Could you check a few things on this model? Use its own coordinates, in mm. A direction names the side the tool comes from. Give positions to 0.01 mm unless a question says otherwise; leave off trailing zeros. Order: outer loops, then holes, each group sorted by start corner. A loop starts at its lowest first (then second) coordinate and runs counter-clockwise, first axis right, second up. Notation, with made-up numbers: (64.25, 48) - (85.25, 48) arc R22 ccw to (85.25, 73) - close; hole circle Ø9 at (32, 82). An arc over 180 degrees is marked (long way). Put each result on its own line as item: value.
from build123d import *

# Parameters (mm, degrees)
CUT_EXTRUDE_START   = -15
CUT_EXTRUDE_1_DEPTH = 4
CHAMFER_1_SIZE      = 1


with BuildPart() as part:
    # 草图1 → 旋转1 (revolve)
    with BuildSketch(Plane.XY, mode=Mode.PRIVATE) as revolve_1_sk:
        Polygon((0, 0), (0, 15), (4.4, 15), (4.4, 14.3), (6, 14.3), (6, 15), (164, 15), (164, 20), (169, 20), (169, 0), align=None)
    revolve(revolve_1_sk.sketch.rotate(Axis((0, 0, 0), (1, 0, 0)), 90), axis=Axis((0, 0, 0), (1, 0, 0)))

    # 草图2 → 切除-拉伸1 (cut)
    with BuildSketch(Plane.XY.offset(CUT_EXTRUDE_START)):
        with BuildLine():
            Line((119, -4), (49, -4))
            ThreePointArc((49, -4), (45, 0), (49, 4))
            Line((49, 4), (119, 4))
            ThreePointArc((119, 4), (123, 0), (119, -4))
        make_face()
    extrude(amount=CUT_EXTRUDE_1_DEPTH, mode=Mode.SUBTRACT)

    # 倒角1
    chamfer_1_edges = [part.edges().sort_by_distance(p)[0] for p in [
        (0, 0, -15),
        (169, 0, -20),
        (164, 0, -20),
    ]]
    chamfer(chamfer_1_edges, length=CHAMFER_1_SIZE)


solid = part.part
1) I'm going to push flat-ended pins straight in: pin 1 (3 mm diameter, centred on x = 100.5, z = -13, fed in from -Y); pin 2 (5 mm diameter, centred on x = 145, y = -11.5, fed in from -Z); pin 3 (4 mm diameter, centred on x = 112.5, z = 15.5, fed in from +Y). Where does each tip first touch, or does it pass through?
Filled in:
pin 1: stops at y = -9.63
pin 2: stops at z = -12
pin 3: stops at y = 6.54
2) Suppose I cut it at A-A, the plane z = 0. List the corners of the cut face in (x, y) for me, and give its area (3 significant figures).
Filled in:
outline: (0, -14) - (1, -15) - (4.4, -15) - (4.4, -14.3) - (6, -14.3) - (6, -15) - (164, -15) - (164, -19) - (165, -20) - (168, -20) - (169, -19) - (169, 19) - (168, 20) - (165, 20) - (164, 19) - (164, 15) - (6, 15) - (6, 14.3) - (4.4, 14.3) - (4.4, 15) - (1, 15) - (0, 14) - close
area: 5,110 mm^2
3) We'd pull the mould along Y, two halves only. Please class faces 4 (the flat face through (84, -4, -13)), 5 (the flat face through (164, -6, -14)), 6 (the cylindrical face through (2.72, -12.65, 8.06)): pulls with the +Y half, pulls with the -Y half, needs draft (parallel to the pull), parting line crosses it, or undercut.
Filled in:
face 4: undercut
face 5: needs draft
face 6: parting line crosses it
4) Suppose I cut it at D-D, the plane x = 62. List the corners of the cut face in (y, z) for me.
Filled in:
outline: (-4, -14.46) - (-4, -11) - (4, -11) - (4, -14.46) arc R15 ccw (long way) to start
5) Suppose I cut it at B-B, the plane y = 0. List the corners of the cut face in (x, z) for me, and give its area (3 significant figures).
Filled in:
outline: (0, -14) - (1, -15) - (4.4, -15) - (4.4, -14.3) - (6, -14.3) - (6, -15) - (45, -15) - (45, -11) - (123, -11) - (123, -15) - (164, -15) - (164, -19) - (165, -20) - (168, -20) - (169, -19) - (169, 19) - (168, 20) - (165, 20) - (164, 19) - (164, 15) - (6, 15) - (6, 14.3) - (4.4, 14.3) - (4.4, 15) - (1, 15) - (0, 14) - close
area: 4,800 mm^2
6) Which directions (+Z, -Z, +X, -X, +Y, -Y) give clear straight access to the entire face, cutting with the end or side of a thin tool? Please do faces 1 (the cylindrical face through (5.21, -14.18, -1.86)), 2 (the cylindrical face through (86.106, -4.506, 14.307)), 3 (the flat face through (84, 4, -13)).
Filled in:
face 1: none
face 2: -X
face 3: -Z
7) If I drill on line 1 (X direction, y = 11.5, z = -9); line 2 (Y direction, x = 91, z = -1); line 3 (X direction, y = 16.5, z = -5.5), over which ranges is the centre line in solid material (lowest first)? Write a range as [from, to].
Filled in:
line 1: x = [0.6, 4.4], [6, 169]
line 2: y = [-14.97, 14.97]
line 3: x = [164, 169]
8) Suppose I cut it at C-C, the plane x = 149.5. List the corners of the cut face in (y, z) for me, and give its area (3 significant figures).
Filled in:
outline: circle Ø30 at (0, 0)
area: 707 mm^2
